from build123d import *

# Parameters (mm, degrees)
SKETCH1_W           = 30
SKETCH1_H           = 30
BOSS_EXTRUDE1_DEPTH = 400
SKETCH2_W           = 24
SKETCH2_H           = 24
CUT_EXTRUDE1_DEPTH  = 492
CUT_EXTRUDE3_DEPTH  = 402.958781438
CUT_EXTRUDE6_DEPTH  = 402.958781438


with BuildPart() as part:
    # Sketch1 → Boss-Extrude1 (new body)
    with BuildSketch(Plane.XY):
        with Locations((-30.141748722, 10.901003365)):
            Rectangle(SKETCH1_W, SKETCH1_H)
    extrude(amount=BOSS_EXTRUDE1_DEPTH)

    # Sketch2 → Cut-Extrude1 (cut)
    with BuildSketch(Plane.XY.offset(400)):
        with Locations((-30.141748722, 10.901003365)):
            Rectangle(SKETCH2_W, SKETCH2_H)
    extrude(amount=-CUT_EXTRUDE1_DEPTH, mode=Mode.SUBTRACT)

    # Sketch4 → Cut-Extrude3 (cut, through all)
    with BuildSketch(Plane(origin=(-15.141748722, 0, 0), x_dir=(0, 0, -1), z_dir=(1, 0, 0))):
        Polygon((0, 25.901003365), (-30, -4.098996635), (0, -4.098996635), align=None)
    extrude(amount=-CUT_EXTRUDE3_DEPTH, mode=Mode.SUBTRACT)

    # Sketch8 → Cut-Extrude6 (cut, through all)
    with BuildSketch(Plane(origin=(-15.141748722, 0, 0), x_dir=(0, 0, -1), z_dir=(1, 0, 0))):
        Polygon((-400, 25.901003365), (-370, -4.098996635), (-400, -4.098996635), align=None)
    extrude(amount=-CUT_EXTRUDE6_DEPTH, mode=Mode.SUBTRACT)


solid = part.part
Read the model definition and answer for the solid it produces. Units are mm, in the model's axes. A direction names the side the tool comes from. Coordinates: 2 decimals unless noted, no trailing zeros. Order: outer loops, then holes, each group sorted by start corner. A loop starts at its lowest first (then second) coordinate and runs counter-clockwise, first axis right, second up. Notation, with made-up numbers: (62, 21) -> (111, 21) arc R27 cw to (111, 37) -> close; hole circle Ø4 at (2.25, 54). An arc over 180 degrees is marked (long way). Answer as a JSON object with one key per item and string values.
1) The mould has two halves that part along Y. Classify faces 3 (the face through (-45.142, 11, 197)), 4 (the face through (-18.142, 11, 203)), 5 (the face through (-43.3, 11.1, 14.8)): released by +Y, released by -Y, zero draft, split by the parting line, or undercut.
Model answer:
{"face 3": "zero draft", "face 4": "undercut", "face 5": "released by -Y"}
2) Consider line 1 along Y through (x, z) = (-33, 207); line 2 along X through (y, z) = (18, 205); line 3 along Z through (x, y) = (-17, 2). Determine where each line is inside the solid, lowest interval first. Write a range as from..to.
Model answer:
{"line 1": "y = -4.1..-1.1, 22.9..25.9", "line 2": "x = -45.14..-42.14, -18.14..-15.14", "line 3": "z = 23.9..376.1"}
3) A tool of negligible diameter and unlimited length cuts with its end or side. For faces 1 (the face through (-42.142, 11, 203)), 2 (the face through (-30, 25.901, 197)), from which of +Z, -Z, +X, -X, +Y, -Y can it reach the whole face along a straight path? Write none if from no direction.
Model answer:
{"face 1": "+Z, -Z", "face 2": "+Z, -Z, +X, -X, +Y"}
4) Each of these flat-tipped pins is pushed along its axis until it touches: pin 1 (10 mm diameter, centred on x = -34.5, y = 17, fed in from +Z); pin 2 (4 mm diameter, centred on x = -41.5, y = 2, fed in from +Z). Where does it stop, or does it pass through?
Model answer:
{"pin 1": "passes through", "pin 2": "stops at z = 377.99"}
5) A cutting plane is placed at C-C, the plane y = 11. Determine the outline of the cut face in (x, z).
Model answer:
{"outline": "(-45.14, 14.9) -> (-42.14, 14.9) -> (-42.14, 385.1) -> (-45.14, 385.1) -> close; (-18.14, 14.9) -> (-15.14, 14.9) -> (-15.14, 385.1) -> (-18.14, 385.1) -> close"}
6) A cutting plane is placed at B-B, the plane z = 288.5. Determine the outline of the cut face in (x, y).
Model answer:
{"outline": "(-45.14, -4.1) -> (-15.14, -4.1) -> (-15.14, 25.9) -> (-45.14, 25.9) -> close; hole (-42.14, -1.1) -> (-18.14, -1.1) -> (-18.14, 22.9) -> (-42.14, 22.9) -> close"}
7) A cutting plane is placed at A-A, the plane x = -37. Determine the outline of the cut face in (y, z).
Model answer:
{"outline": "(-4.1, 30) -> (-1.1, 27) -> (-1.1, 373) -> (-4.1, 370) -> close; (22.9, 3) -> (25.9, 0) -> (25.9, 400) -> (22.9, 397) -> close"}
